The listing builds one solid part. Answer for the finished solid, in the listing's coordinates (mm). Face numbers are marked on the shaded views. A direction names the side the tool comes from. Round coordinates to 2 decimals unless told otherwise and drop trailing zeros. Loops run counter-clockwise (first coordinate to the right, second up) from the corner with the lowest first, then second, coordinate; pieces in that order, holes last. Notation, with made-up numbers: M 59.5,86.25 L 92.5,86.25 A21 cw 92.5,108.25 Z; hole C 68,-7.5 d6. An arc over 180 degrees is marked long. Put each result on its own line as item: value. Start each with the question number.
(1) Section B-B, the plane y = 45 is taken. Determine the outline of the cut face in (x, z).
(2) Determine the mould class of the marked faces 6, 7 and 8 for opening direction X: released by +X, released by -X, zero draft, split by the parting line, or undercut.
(3) Section C-C, the plane z = -40 is taken. Determine the outline of the cut face in (x, y), then the cut area to 3 significant figures.
(4) Straight lines are drawn through the part: line 1 (Z direction, x = 23, y = 5.5); line 2 (Y direction, x = 39, z = -40); line 3 (Z direction, x = 16.5, y = 49). For each, find the intervals that lie inside material, in ascending order.
(5) Flat-ended cylindrical pins translate along their axes: P1, Ø10, axis at y = 44, z = -67.5, coming from the +X side; P2, Ø3, axis at x = 5, z = -55, coming from the +Y side; P3, Ø3.5, axis at x = 22, y = 4.5, coming from the +Z side; P4, Ø7, axis at x = 16.5, y = 21.5, coming from the -Z side. Find the tip coordinate at first contact, or state that the pin passes through.
(6) Section D-D, the plane y = 5.5 is taken. Determine the outline of the cut face in (x, z), then the cut area to 3 significant figures.
(7) Section A-A, the plane x = 15 is taken. Determine the outline of the cut face in (y, z), then the cut area to 3 significant figures.
(8) Which of the six approach directions +Z, -Z, +X, -X, +Y, -Y give full straight-line access (tool end or side, diameter ignored) to the marked faces 1, 2, 3, 4 and 5?
```python
from build123d import *

# Parameters (mm, degrees)
BASE_PLATE_DEPTH             = 46
HUB_PROFILE_36_18_R          = 18
HUB_PROFILE_36_18_R_2        = 9
BEARING_HUB_36_BORE_18_DEPTH = 50
HUB_SUPPORT_WEB_REACH        = 109.243
HUB_SUPPORT_WEB_END_RADIUS   = 18
HUB_SUPPORT_PROFILE_W        = 36
HUB_SUPPORT_PROFILE_H        = 12
MOUNTING_SLOTS_2X_DEPTH      = 108.24271537
EDGE_FILLETS_R2_5_R          = 2.5


with BuildPart() as part:
    # Base Plate Profile → Base Plate (new body)
    with BuildSketch(Plane(origin=(0, 0, 0), x_dir=(0, 0, -1), z_dir=(1, 0, 0))):
        Polygon((0, 0), (30, 0), (30, -3), (50, -3), (50, 0), (80, 0), (80, 12), (0, 12), align=None)
    extrude(amount=BASE_PLATE_DEPTH)



with BuildPart() as body_2:
    # Hub Profile Ø36-Ø18 → Bearing Hub Ø36 Bore Ø18 (new body)
    with BuildSketch(Plane.ZY):
        with Locations((-40, 45)):
            Circle(HUB_PROFILE_36_18_R)
        with Locations((-40, 45)):
            Circle(HUB_PROFILE_36_18_R_2, mode=Mode.SUBTRACT)
    extrude(amount=-BEARING_HUB_36_BORE_18_DEPTH)


with BuildPart() as part_1:
    add(part.part)

    add(body_2.part)  # Hub Support Web merges body 2
    # Hub Support Web: up to this cylinder (the profile starts outside it)
    hub_support_web_end = Plane(origin=(25, 45, -40), z_dir=(-1, 0, 0)) * Cylinder(HUB_SUPPORT_WEB_END_RADIUS, 255.486, mode=Mode.PRIVATE)
    # Hub Support Profile → Hub Support Web (add, up to the surface)
    with BuildSketch(Plane(origin=(0, 12, 0), x_dir=(1, 0, 0), z_dir=(0, 1, 0)), mode=Mode.PRIVATE) as hub_support_web_sk1:
        with Locations((25, 40)):
            Rectangle(HUB_SUPPORT_PROFILE_W, HUB_SUPPORT_PROFILE_H)
    hub_support_web_tool1 = extrude(hub_support_web_sk1.sketch, amount=HUB_SUPPORT_WEB_REACH, mode=Mode.PRIVATE) - hub_support_web_end
    add(hub_support_web_tool1.solids().sort_by_distance((25, 12, -40))[0])

    # Mounting Slots Profile → Mounting Slots 2x (cut, through all)
    with BuildSketch(Plane(origin=(0, 12, 0), x_dir=(1, 0, 0), z_dir=(0, 1, 0))):
        with BuildLine():
            Line((13, 76.385225424), (33, 76.385225424))
            ThreePointArc((33, 76.385225424), (38, 71.385225424), (33, 66.385225424))
            Line((33, 66.385225424), (13, 66.385225424))
            ThreePointArc((13, 66.385225424), (8, 71.385225424), (13, 76.385225424))
        make_face()
        with BuildLine():
            Line((13, 14.243278019), (33, 14.243278019))
            ThreePointArc((33, 14.243278019), (38, 9.243278019), (33, 4.243278019))
            Line((33, 4.243278019), (13, 4.243278019))
            ThreePointArc((13, 4.243278019), (8, 9.243278019), (13, 14.243278019))
        make_face()
    extrude(amount=-MOUNTING_SLOTS_2X_DEPTH, mode=Mode.SUBTRACT)

    # Edge Fillets R2.5
    edge_fillets_r2_5_edges = [part_1.edges().sort_by_distance(p)[0] for p in [
        (25, 12, -34),
        (7, 12, -40),
        (25, 12, -46),
        (43, 12, -40),
    ]]
    fillet(edge_fillets_r2_5_edges, radius=EDGE_FILLETS_R2_5_R)


solid = part_1.part
```
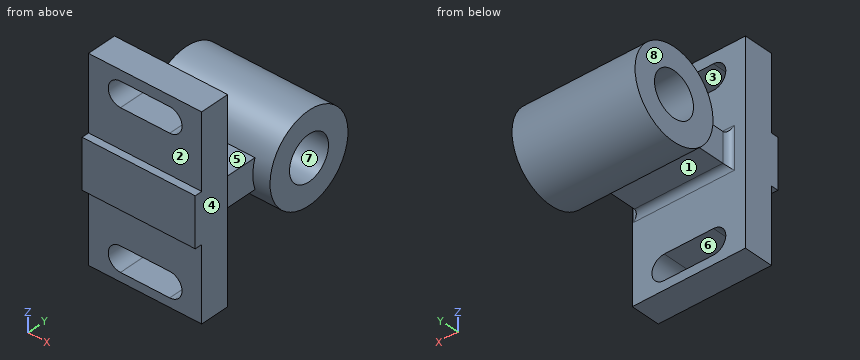
Recorded:
1. outline: M 0,-58 L 50,-58 L 50,-49 L 0,-49 Z; M 0,-31 L 50,-31 L 50,-22 L 0,-22 Z
2. face 6: undercut
2. face 7: zero draft
2. face 8: released by -X
3. outline: M 0,-3 L 46,-3 L 46,12 L 45.5,12 A2.5 cw 43,14.5 L 43,27 L 50,27 L 50,36 L 0,36 L 0,27 L 7,27 L 7,14.5 A2.5 cw 4.5,12 L 0,12 Z; M 0,54 L 50,54 L 50,63 L 0,63 Z
3. area: 2,130 mm²
4. line 1: z = -80 to -76.39, -66.39 to -14.24, -4.24 to 0
4. line 2: y = -3 to 36, 54 to 63
4. line 3: z = -57.55 to -48.06, -31.94 to -22.45
5. P1: passes through
5. P2: stops at y = 56.91
5. P3: stops at z = 0
5. P4: stops at z = -46
6. outline: M 0,-80 L 46,-80 L 46,0 L 0,0 Z; hole M 13,-76.39 L 33,-76.39 A5 ccw 33,-66.39 L 13,-66.39 A5 ccw Z; hole M 13,-14.24 L 33,-14.24 A5 ccw 33,-4.24 L 13,-4.24 A5 ccw Z
6. area: 3,120 mm²
7. outline: M -3,-50 L 0,-50 L 0,-66.39 L 12,-66.39 L 12,-48.5 A2.5 cw 14.5,-46 L 28.03,-46 A18 ccw long 28.03,-34 L 14.5,-34 A2.5 cw 12,-31.5 L 12,-14.24 L 0,-14.24 L 0,-30 L -3,-30 Z; M 0,-80 L 12,-80 L 12,-76.39 L 0,-76.39 Z; M 0,-4.24 L 12,-4.24 L 12,0 L 0,0 Z; hole C 45,-40 d18
7. area: 1,730 mm²
8. face 1: -Z, +X, -X
8. face 2: +Z, +X, -X, -Y
8. face 3: +Y, -Y
8. face 4: +Z, -Z, +X, -Y
8. face 5: +Z, +X, -X
